Print and shaded views of the part. All mm, measured from the part's lowest x, y and z. Give positions to 0.01 mm unless a question says otherwise; leave off trailing zeros. Loops run counter-clockwise (first coordinate to the right, second up) from the corner with the lowest first, then second, coordinate; pieces in that order, holes last.
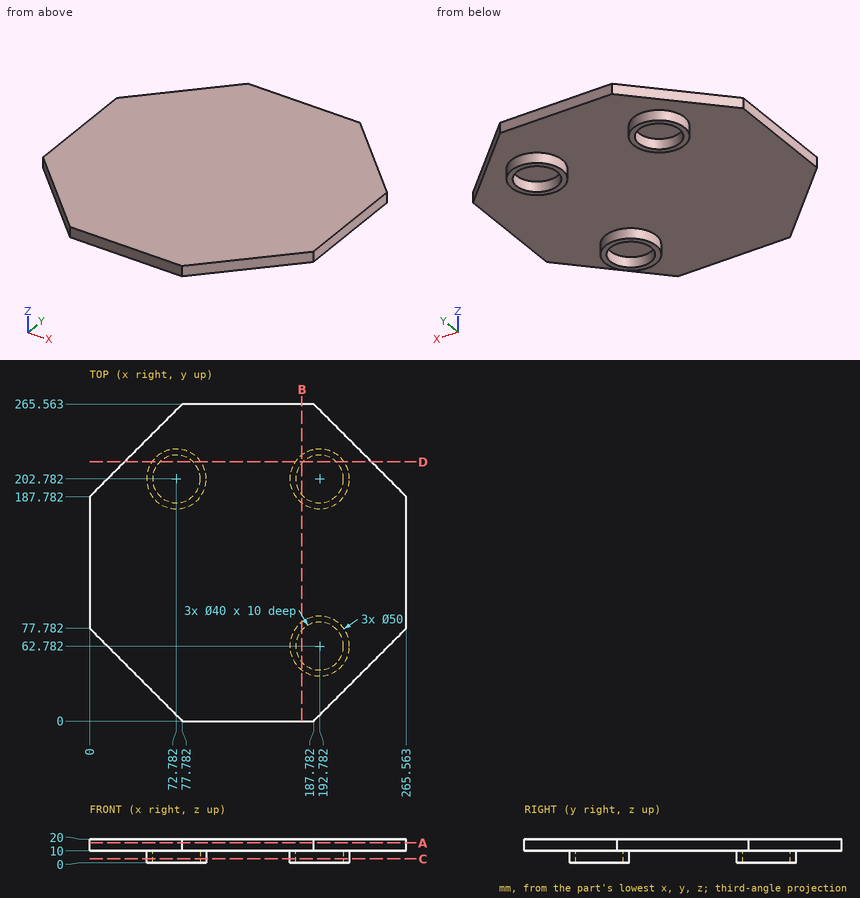
1. Saw through at B-B, the plane x = 178. List the corners of the cut face in (y, z), and give its area (3 significant figures).
Responses:
outline: (0, 10) - (42.62, 10) - (42.62, 0) - (49.31, 0) - (49.31, 10) - (76.25, 10) - (76.25, 0) - (82.94, 0) - (82.94, 10) - (182.62, 10) - (182.62, 0) - (189.31, 0) - (189.31, 10) - (216.25, 10) - (216.25, 0) - (222.94, 0) - (222.94, 10) - (265.56, 10) - (265.56, 20) - (0, 20) - close
area: 2,920 mm2
2. Saw through at C-C, the plane z = 3.25. List the corners of the cut face in (x, y), and give its area (3 significant figures).
Responses:
outline: circle Ø50 at (72.78, 202.78); circle Ø50 at (192.78, 62.78); circle Ø50 at (192.78, 202.78); hole circle Ø40 at (72.78, 202.78); hole circle Ø40 at (192.78, 62.78); hole circle Ø40 at (192.78, 202.78)
area: 2,120 mm2
3. Drop flat-ended pins along their axis: pin 1 (5 mm diameter, centred on y = 40.5, z = 5, fed in from +X); pin 2 (12 mm diameter, centred on x = 188.5, y = 58.5, fed in from -Z); pin 3 (6 mm diameter, centred on y = 46.5, z = 10.5, fed in from +X). Give the stop position or say it passes through.
Responses:
pin 1: stops at x = 208.07
pin 2: stops at z = 10
pin 3: stops at x = 237.28
4. Saw through at D-D, the plane y = 217. List the corners of the cut face in (x, z) (1 decimal).
Responses:
outline: (29.2, 10) - (52.2, 10) - (52.2, 0) - (58.7, 0) - (58.7, 10) - (86.8, 10) - (86.8, 0) - (93.3, 0) - (93.3, 10) - (172.2, 10) - (172.2, 0) - (178.7, 0) - (178.7, 10) - (206.8, 10) - (206.8, 0) - (213.3, 0) - (213.3, 10) - (236.3, 10) - (236.3, 20) - (29.2, 20) - close
5. Probe line 1 along Z through (x, y) = (113, 168.5); line 2 along Y through (x, z) = (60, 1) (1 decimal); line 3 along Y through (x, z) = (67, 6.5) (1 decimal). List the from-to ranges inside material, lowest first.
Responses:
line 1: z = 10 to 20
line 2: y = 181.3 to 187.4, 218.2 to 224.3
line 3: y = 178.5 to 183.6, 221.9 to 227.1
6. Saw through at A-A, the plane z = 16.75. List the corners of the cut face in (x, y), and give its area (3 significant figures).
Responses:
outline: (0, 77.78) - (77.78, 0) - (187.78, 0) - (265.56, 77.78) - (265.56, 187.78) - (187.78, 265.56) - (77.78, 265.56) - (0, 187.78) - close
area: 58,400 mm2
